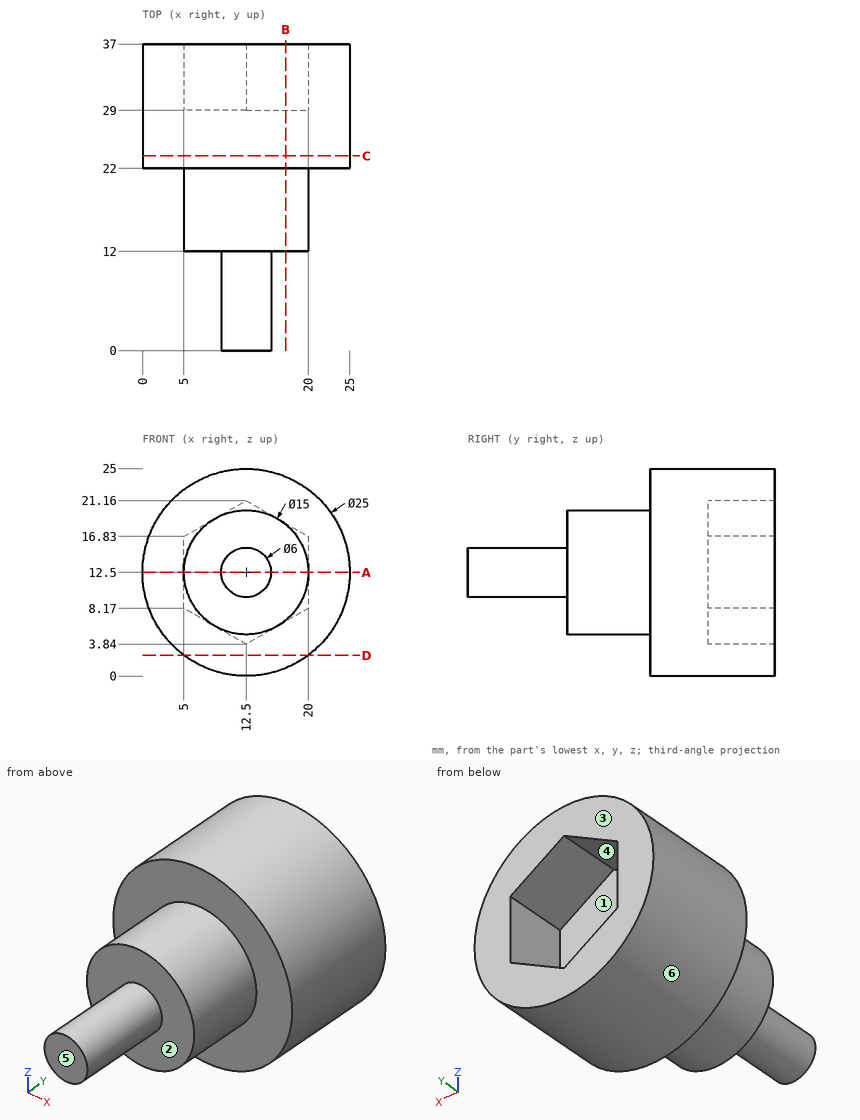
Study the drawing (mm; zero at the part's minimum x, y, z) and answer. A direction names the side the tool comes from. Round coordinates to 2 decimals unless told otherwise and drop trailing zeros. Loops run counter-clockwise (first coordinate to the right, second up) from the corner with the lowest first, then second, coordinate; pieces in that order, holes last. Notation, with made-up numbers: (17.25, -22) -> (30.25, -22) arc R13 ccw to (30.25, -14) -> close; hole circle Ø11 at (29, -29.5). An arc over 180 degrees is marked (long way). One line per item, written item: value.
1) The mould has two halves that part along X. Classify the marked faces 4, 5 and 6: pulls with the +X half, pulls with the -X half, needs draft (parallel to the pull), parting line crosses it, or undercut.
Answer list:
face 4: undercut
face 5: needs draft
face 6: parting line crosses it
2) For the marked faces 1, 2 and 3, determine the directions among +Z, -Z, +X, -X, +Y, -Y from which every point of the face is accessible in a straight line to the end or side of a thin tool.
Answer list:
face 1: +Y
face 2: -Y
face 3: +Z, -Z, +X, -X, +Y
3) Consider L1, parallel to Y at x = 16.25, z = 9.5; L2, parallel to Z at x = 12.25, y = 6; L3, parallel to Y at x = 14, z = 2.75. Determine where each line is inside the solid, lowest interval first. Write a range as [from, to].
Answer list:
L1: y = [12, 29]
L2: z = [9.51, 15.49]
L3: y = [22, 37]
4) A cutting plane is placed at D-D (z = 2.5). Determine the outline of the cut face in (x, y), and give its area (3 significant figures).
Answer list:
outline: (5, 22) -> (20, 22) -> (20, 37) -> (5, 37) -> close
area: 225 mm²
5) A cutting plane is placed at B-B (x = 17.25). Determine the outline of the cut face in (y, z).
Answer list:
outline: (12, 6.7) -> (22, 6.7) -> (22, 0.94) -> (37, 0.94) -> (37, 6.58) -> (29, 6.58) -> (29, 18.42) -> (37, 18.42) -> (37, 24.06) -> (22, 24.06) -> (22, 18.3) -> (12, 18.3) -> close
6) A cutting plane is placed at A-A (z = 12.5). Determine the outline of the cut face in (x, y), and give its area (3 significant figures).
Answer list:
outline: (0, 22) -> (5, 22) -> (5, 12) -> (9.5, 12) -> (9.5, 0) -> (15.5, 0) -> (15.5, 12) -> (20, 12) -> (20, 22) -> (25, 22) -> (25, 37) -> (20, 37) -> (20, 29) -> (5, 29) -> (5, 37) -> (0, 37) -> close
area: 477 mm²
7) Flat-ended cylindrical pins translate along their axes: P1, Ø10, axis at x = 19.5, y = 31, coming from the -Z side; P2, Ø7.5, axis at x = 13.5, z = 12.5, coming from the -Y side; P3, Ø4, axis at x = 19, y = 18, coming from the +Z side; P4, Ø4, axis at y = 6.5, z = 8, coming from the +X side. Find the tip coordinate at first contact, or state that the pin passes through.
Answer list:
P1: stops at z = 0.16
P2: stops at y = 0
P3: stops at z = 18.5
P4: stops at x = 14.16
8) A cutting plane is placed at C-C (y = 23.5). Determine the outline of the cut face in (x, z), and give its area (3 significant figures).
Answer list:
outline: circle Ø25 at (12.5, 12.5)
area: 491 mm²
